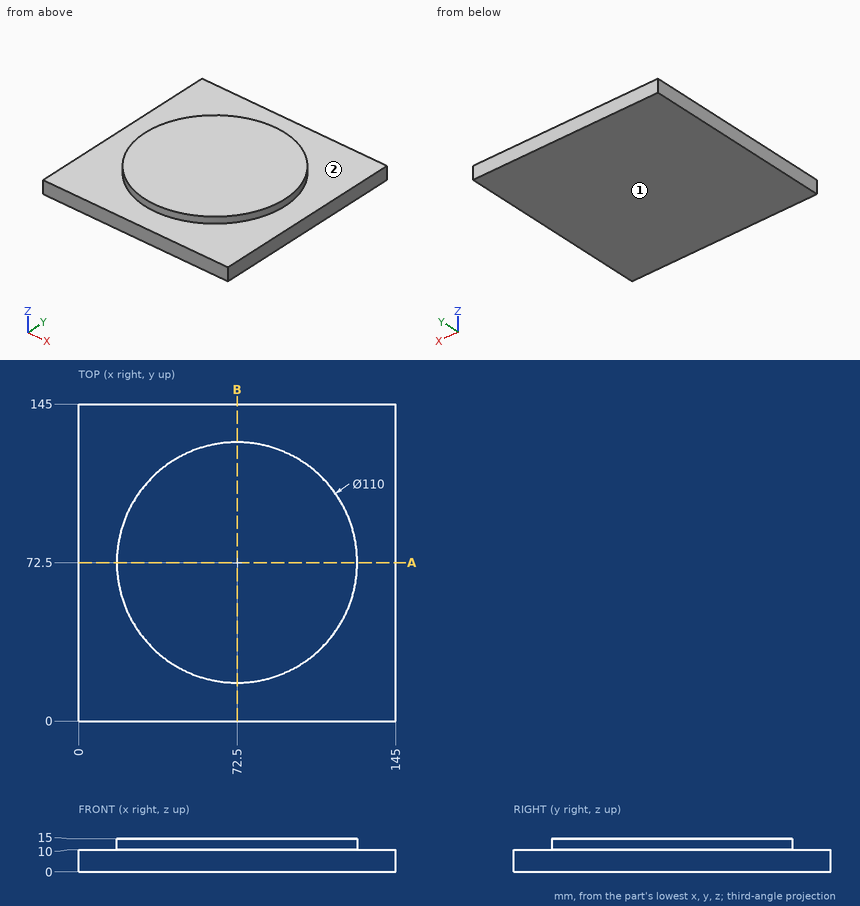
Could you check a few things on this drawing? It's one solid part, dimensions in mm from its lowest x, y, z. A direction names the side the tool comes from. Coordinates: 2 decimals unless noted, no trailing zeros. Order: outer loops, then holes, each group sorted by start corner. A loop starts at its lowest first (then second) coordinate and runs counter-clockwise, first axis right, second up. Notation, with made-up numbers: (-35.5, -7) - (-30.5, -7) arc R21 ccw to (-30.5, 8) - close; hole circle Ø9 at (9.5, 38.25). An arc over 180 degrees is marked (long way). Answer as a JSON object with one key per item and string values. Group by question number.
Q1. Will this pin go through, and if not, where does the flat tip stop? P1, Ø1, axis at x = 35, z = 13, coming from the -Y side.
Q2. On a 3-axis mill with a long thin cutter (end or side, diameter ignored), from which of +Z, -Z, +X, -X, +Y, -Y can I reach the whole of each face in a straight line? I mean the marked faces 1 and 2. Say none if no direction works.
Q3. Imagine slicing it at A-A (y = 72.5). Please give me the cut outline in (x, z).
Q4. I need wall thicknesses on line 1 (Z direction, x = 138.5, y = 136); line 2 (X direction, y = 116.5, z = 14); line 3 (X direction, y = 21.5, z = 11.75). Which ranges of each line are inside material? Lowest first, please. Write a range as from..to.
Determined:
{
 "1": {"P1": "stops at y = 31.81"},
 "2": {"face 1": "-Z, +X, -X, +Y, -Y", "face 2": "+Z"},
 "3": {"outline": "(0, 0) - (145, 0) - (145, 10) - (127.5, 10) - (127.5, 15) - (17.5, 15) - (17.5, 10) - (0, 10) - close"},
 "4": {"line 1": "z = 0..10", "line 2": "x = 39.5..105.5", "line 3": "x = 51.91..93.09"}
}
